For this review, use the dimensioned drawing (mm, ordinates from the lowest corner) and the shaded views. A direction names the side the tool comes from. Give positions to 0.01 mm unless a question says otherwise; leave off trailing zeros. Loops run counter-clockwise (first coordinate to the right, second up) from the corner with the lowest first, then second, coordinate; pieces in that order, holes last. Notation, with made-up numbers: (84.25, 46.5) - (123.25, 46.5) arc R17 cw to (123.25, 56.5) - close; hole circle Ø4 at (18, 30.25). An arc over 180 degrees is marked (long way). Write each question's results on one line, items separated by ' | '.
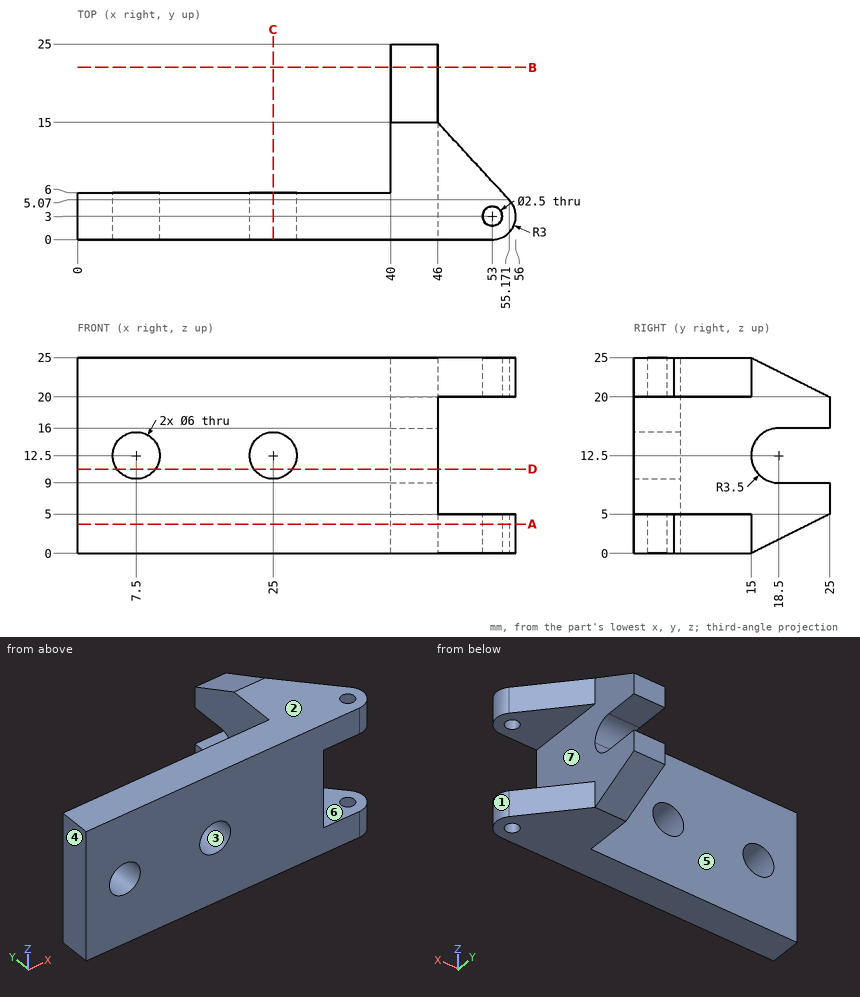
Item 1: Wall thickness on probe 1 along X at (y, z) = (3, 12.5); probe 2 along X at (y, z) = (3, 13.5); probe 3 along Y at (x, z) = (29, 23.5): over which ranges is each line inside the solid? List them lowest first.
Output values:
probe 1: x = 0 to 4.5, 10.5 to 22, 28 to 46 | probe 2: x = 0 to 4.67, 10.33 to 22.17, 27.83 to 46 | probe 3: y = 0 to 6
Item 2: Tool access review of the marked faces 5, 6 and 7: name each direction out of +Z, -Z, +X, -X, +Y, -Y from which nothing blocks a thin tool from reaching the whole face with its end or side.
Output values:
face 5: +Z, -Z, -X, +Y | face 6: +X, +Y, -Y | face 7: +X, +Y
Item 3: We need section C-C on x = 25. Give the boundary of the cut face in (y, z), then the cut area to 3 significant figures.
Output values:
outline: (0, 0) - (6, 0) - (6, 9.5) - (0, 9.5) - close; (0, 15.5) - (6, 15.5) - (6, 25) - (0, 25) - close | area: 114 mm²
Item 4: We need section B-B on y = 22. Give the boundary of the cut face in (x, z).
Output values:
outline: (40, 3.5) - (46, 3.5) - (46, 9) - (40, 9) - close; (40, 16) - (46, 16) - (46, 21.5) - (40, 21.5) - close
Item 5: We need section D-D on z = 10.75. Give the boundary of the cut face in (x, y).
Output values:
outline: (0, 0) - (5.06, 0) - (5.06, 6) - (0, 6) - close; (9.94, 0) - (22.56, 0) - (22.56, 6) - (9.94, 6) - close; (27.44, 0) - (46, 0) - (46, 15.47) - (40, 15.47) - (40, 6) - (27.44, 6) - close
Item 6: Clearance check with flat-ended pins moving along their axes: P1, Ø1, axis at y = 20.5, z = 20, coming from the +X side; P2, Ø5, axis at x = 42, y = 21.5, coming from the +Z side; P3, Ø6, axis at y = 12.5, z = 20, coming from the -X side. State where each tip first meets the part, or that it passes through.
Output values:
P1: stops at x = 46 | P2: stops at z = 23 | P3: stops at x = 40
Item 7: We need section A-A on z = 3.75. Give the boundary of the cut face in (x, y).
Output values:
outline: (0, 0) - (53, 0) arc R3 ccw to (55.17, 5.07) - (46, 15) - (46, 22.5) - (40, 22.5) - (40, 6) - (0, 6) - close; hole circle Ø2.5 at (53, 3)
Item 8: Draft analysis for pull direction X (two halves, no side actions). For the marked faces 1, 2, 3 and 4, state which applies: +X half, -X half, draft (parallel to the pull), parting line (faces both ways), or undercut.
Output values:
face 1: +X half | face 2: draft | face 3: undercut | face 4: -X half
